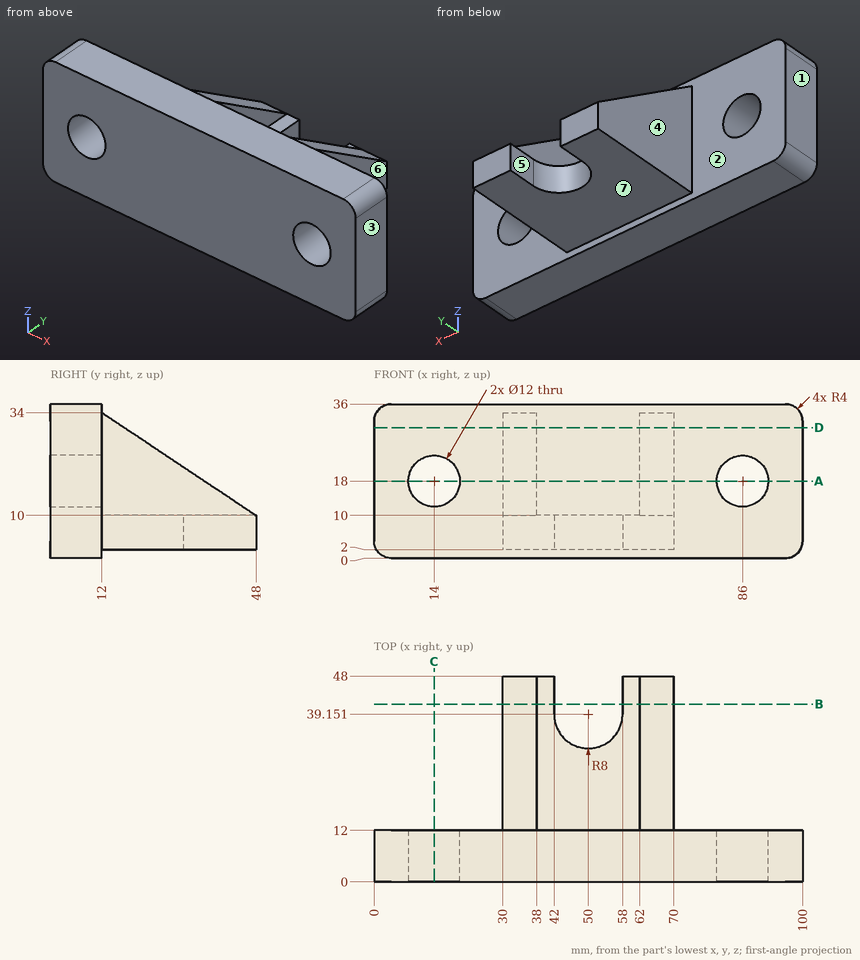
The figure shows three views and two pictorial views of one solid part (mm, origin at its lowest corner). Answer the questions. A direction names the side the tool comes from. Round coordinates to 2 decimals unless told otherwise and drop trailing zeros. Loops run counter-clockwise (first coordinate to the right, second up) from the corner with the lowest first, then second, coordinate; pieces in that order, holes last. Notation, with made-up numbers: M 18.25,8.25 L 41.25,8.25 A14 cw 41.25,27.25 Z; hole C -13.5,23.5 d10. An arc over 180 degrees is marked long. Write each question's results on one line, items separated by ' | '. Start each with the question number.
1) Find section D-D on z = 30.5. Write down the section's boundary in (x, y).
2) Find section B-B on y = 41.5. Write down the section's boundary in (x, z).
3) Straight lines are drawn through the part: probe 1 along X at (y, z) = (41.5, 2.5); probe 2 along Z at (x, y) = (14, 7); probe 3 along Y at (x, z) = (27, 9). For each, find the intervals that lie inside material, in ascending order.
4) Each of these flat-tipped pins is pushed along its axis until it touches: pin 1 (7 mm diameter, centred on y = 38.5, z = 18.5, fed in from +X); pin 2 (2.5 mm diameter, centred on y = 44, z = 8, fed in from -X); pin 3 (12 mm diameter, centred on x = 51.5, y = 34.5, fed in from +Z). Where does it stop, or does it pass through?
5) Find section C-C on x = 14. Write down the section's boundary in (y, z), plus the area to 3 significant figures.
6) Which of the six approach directions +Z, -Z, +X, -X, +Y, -Y give full straight-line access (tool end or side, diameter ignored) to the marked faces 4, 5, 6 and 7?
7) Determine the mould class of the marked faces 1, 2 and 3 for opening direction X: pulls with the +X half, pulls with the -X half, needs draft (parallel to the pull), parting line crosses it, or undercut.
8) Find section A-A on z = 18. Write down the section's boundary in (x, y).
Final values:
1) outline: M 0,0 L 100,0 L 100,12 L 70,12 L 70,17.25 L 62,17.25 L 62,12 L 38,12 L 38,17.25 L 30,17.25 L 30,12 L 0,12 Z
2) outline: M 30,2 L 42,2 L 42,10 L 38,10 L 38,14.33 L 30,14.33 Z; M 58,2 L 70,2 L 70,14.33 L 62,14.33 L 62,10 L 58,10 Z
3) probe 1: 30 to 42, 58 to 70 | probe 2: 0 to 12, 24 to 36 | probe 3: 0 to 12
4) pin 1: x = 70 | pin 2: x = 30 | pin 3: z = 10
5) outline: M 0,0 L 12,0 L 12,12 L 0,12 Z; M 0,24 L 12,24 L 12,36 L 0,36 Z | area: 288 mm²
6) face 4: +Z, -Z, -X, +Y | face 5: +Z, -Z, +Y | face 6: +Z, -Z, +X, +Y | face 7: -Z, +X, -X, +Y
7) face 1: pulls with the -X half | face 2: undercut | face 3: pulls with the +X half
8) outline: M 0,0 L 8,0 L 8,12 L 0,12 Z; M 20,0 L 80,0 L 80,12 L 70,12 L 70,36 L 62,36 L 62,12 L 38,12 L 38,36 L 30,36 L 30,12 L 20,12 Z; M 92,0 L 100,0 L 100,12 L 92,12 Z
